Read the model definition and answer for the solid it produces. Units are mm, in the model's axes. A direction names the side the tool comes from. Round coordinates to 2 decimals unless told otherwise and drop trailing zeros. Order: outer loops, then holes, each group sorted by start corner. A loop starts at its lowest first (then second) coordinate and runs counter-clockwise, first axis right, second up. Notation, with made-up numbers: (59.5, 60) - (89.5, 60) arc R24 cw to (89.5, 98) - close; hole circle Ø11 at (22.5, -17). An arc over 180 degrees is marked (long way). Answer as a JSON object with one key per item and string values. Group by question number.
Q1. A cutting plane is placed at D-D on z = -9. Determine the outline of the cut face in (x, y), and give its area (3 significant figures).
Q2. Consider line 1 (Y direction, x = 2.75, z = -48); line 2 (Z direction, x = 9, y = 14); line 3 (Y direction, x = 5.25, z = -4.5). Determine where each line is inside the solid, lowest interval first.
Q3. A cutting plane is placed at C-C on z = -48. Determine the outline of the cut face in (x, y).
Q4. A cutting plane is placed at B-B on y = 0. Determine the outline of the cut face in (x, z).
Q5. Given pin 1 Ø5.5 at (y, z) = (14.85, -62.85) entering from -X; pin 2 Ø2 at (x, z) = (2.5, -57.5) entering from -Y; pin 3 Ø4 at (x, z) = (4, -47.5) entering from +Y; pin 4 Ø5 at (x, y) = (7.5, -35) entering from -Z, each flat-ended and moving along its own axis, determine where each tip first touches the part or whether it passes through.
Q6. A tool of negligible diameter and unlimited length cuts with its end or side. For faces 5 (the flat face through (4, 35, -10)), 6 (the cylindrical face through (4.93, -13.734, -64.065)), 7 (the flat face through (5, -21, -42)), from which of +Z, -Z, +X, -X, +Y, -Y can it reach the whole face along a straight path? Write none if from no direction.
Q7. A cutting plane is placed at A-A on x = 5.25. Determine the outline of the cut face in (y, z), and give its area (3 significant figures).
Q8. The mould has two halves that part along Z. Classify faces 1 (the flat face through (5, 21, -42)), 2 (the flat face through (5, -1, 0)), 3 (the flat face through (2.7, -34.5, -10)), 4 (the cylindrical face through (4.9, 14.9, -64.5)): pulls with the +Z half, pulls with the -Z half, needs draft (parallel to the pull), parting line crosses it, or undercut.
```python
from build123d import *

# Parameters (mm, degrees)
BOSS_EXTRUDE1_DEPTH        = 10
SKETCH2_R                  = 17
CUT_EXTRUDE1_DEPTH         = 81.380345856
F_5_5_5_5_DIAMETER_HOLE1_D = 5.5
M4_TAPPED_HOLE1_D          = 3.3
FILLET1_R                  = 5
CHAMFER1_SIZE              = 0.5


with BuildPart() as part:
    # Sketch1 → Boss-Extrude1 (new body)
    with BuildSketch(Plane(origin=(0, 0, 0), x_dir=(0, 0, -1), z_dir=(1, 0, 0))):
        Polygon((0, -40), (0, 40), (10, 40), (10, 21), (69, 21), (69, -21), (10, -21), (10, -40), align=None)
    extrude(amount=BOSS_EXTRUDE1_DEPTH)

    # Sketch2 → Cut-Extrude1 (cut, through all)
    with BuildSketch(Plane(origin=(10, 0, 0), x_dir=(0, 0, -1), z_dir=(1, 0, 0))):
        with Locations((48, 0)):
            Circle(SKETCH2_R)
    extrude(amount=-CUT_EXTRUDE1_DEPTH, mode=Mode.SUBTRACT)

    # Ø5.5 (5.5) Diameter Hole1 (through all)
    with Locations(Plane.XY):
        with Locations((5, 32), (5, -32)):
            Hole(F_5_5_5_5_DIAMETER_HOLE1_D / 2)

    # M4 Tapped Hole1 (through all)
    with Locations(Plane(origin=(10, 0, 0), x_dir=(0, 0, -1), z_dir=(1, 0, 0))):
        with Locations((33.150757595, 14.849242405), (62.849242405, 14.849242405), (62.849242405, -14.849242405), (33.150757595, -14.849242405)):
            Hole(M4_TAPPED_HOLE1_D / 2)

    # Fillet1
    fillet1_edges = [part.edges().sort_by_distance(p)[0] for p in [
        (5, 21, -10),
        (5, -21, -10),
    ]]
    fillet(fillet1_edges, radius=FILLET1_R)

    # Chamfer1
    chamfer1_edges = [part.edges().sort_by_distance(p)[0] for p in [
        (0, 0, -31),
        (10, 0, -31),
    ]]
    chamfer(chamfer1_edges, length=CHAMFER1_SIZE)


solid = part.part
```
Result set:
{
 "1": {"outline": "(0, -40) - (10, -40) - (10, 40) - (0, 40) - close; hole circle Ø5.5 at (5, -32); hole circle Ø5.5 at (5, 32)", "area": "752 mm²"},
 "2": {"line 1": "y = -21 to -17, 17 to 21", "line 2": "z = -69 to -64.26, -61.43 to -57.64, -38.36 to -34.57, -31.74 to 0", "line 3": "y = -40 to -34.74, -29.26 to 29.26, 34.74 to 40"},
 "3": {"outline": "(0, -21) - (10, -21) - (10, -17.5) - (9.5, -17) - (0.5, -17) - (0, -17.5) - close; (0, 17.5) - (0.5, 17) - (9.5, 17) - (10, 17.5) - (10, 21) - (0, 21) - close"},
 "4": {"outline": "(0, -69) - (10, -69) - (10, -65.5) - (9.5, -65) - (0.5, -65) - (0, -65.5) - close; (0, -30.5) - (0.5, -31) - (9.5, -31) - (10, -30.5) - (10, 0) - (0, 0) - close"},
 "5": {"pin 1": "stops at x = 0", "pin 2": "stops at y = -21", "pin 3": "stops at y = 21", "pin 4": "stops at z = -10"},
 "6": {"face 5": "-Z, +X, -X, +Y", "face 6": "+X, -X", "face 7": "-Z, +X, -X, -Y"},
 "7": {"outline": "(-40, -10) - (-34.74, -10) - (-34.74, 0) - (-40, 0) - close; (-29.26, -10) - (-26, -10) arc R5 cw to (-21, -15) - (-21, -69) - (21, -69) - (21, -15) arc R5 cw to (26, -10) - (29.26, -10) - (29.26, 0) - (-29.26, 0) - close; (34.74, -10) - (40, -10) - (40, 0) - (34.74, 0) - close; hole circle Ø34 at (0, -48); hole circle Ø3.3 at (-14.85, -62.85); hole circle Ø3.3 at (-14.85, -33.15); hole circle Ø3.3 at (14.85, -62.85); hole circle Ø3.3 at (14.85, -33.15)", "area": "2,240 mm²"},
 "8": {"face 1": "needs draft", "face 2": "pulls with the +Z half", "face 3": "pulls with the -Z half", "face 4": "undercut"}
}
